For this review, take the finished solid that the model builds, in its own axes (mm). Face numbers are marked on the shaded views. A direction names the side the tool comes from. Give positions to 0.01 mm unless a question says otherwise; leave off trailing zeros. Write each loop counter-clockwise with the first axis right and the second up, starting at its lowest first coordinate (ties: lowest second). Pieces come first, ordered by that corner, then holes.
from build123d import *

# Parameters (mm, degrees)
SKETCH1_W           = 80
SKETCH1_H           = 30
SKETCH1_R           = 5.5
BOSS_EXTRUDE1_DEPTH = 6
SKETCH3_W           = 50
SKETCH3_H           = 30
SKETCH3_R           = 5
BOSS_EXTRUDE2_DEPTH = 6
FILLET1_R           = 2
CHAMFER1_SIZE       = 5


with BuildPart() as part:
    # Sketch1 → Boss-Extrude1 (new body)
    with BuildSketch(Plane.XY):
        Rectangle(SKETCH1_W, SKETCH1_H)
        Circle(SKETCH1_R, mode=Mode.SUBTRACT)
        with Locations((-25, 0)):
            Circle(SKETCH1_R, mode=Mode.SUBTRACT)
    extrude(amount=BOSS_EXTRUDE1_DEPTH)

    # Sketch3 → Boss-Extrude2 (add)
    with BuildSketch(Plane(origin=(40, 0, 0), x_dir=(0, 0, -1), z_dir=(1, 0, 0))):
        with Locations((-25, 0)):
            Rectangle(SKETCH3_W, SKETCH3_H)
        with Locations((-40, 0)):
            Circle(SKETCH3_R, mode=Mode.SUBTRACT)
    extrude(amount=-BOSS_EXTRUDE2_DEPTH)

    # Fillet1
    fillet1_edges = [part.edges().sort_by_distance(p)[0] for p in [
        (34, 0, 6),
        (40, 0, 0),
    ]]
    fillet(fillet1_edges, radius=FILLET1_R)

    # Chamfer1
    chamfer1_edges = [part.edges().sort_by_distance(p)[0] for p in [
        (37, 15, 50),
        (37, -15, 50),
        (-40, -15, 3),
        (-40, 15, 3),
    ]]
    chamfer(chamfer1_edges, length=CHAMFER1_SIZE)


solid = part.part
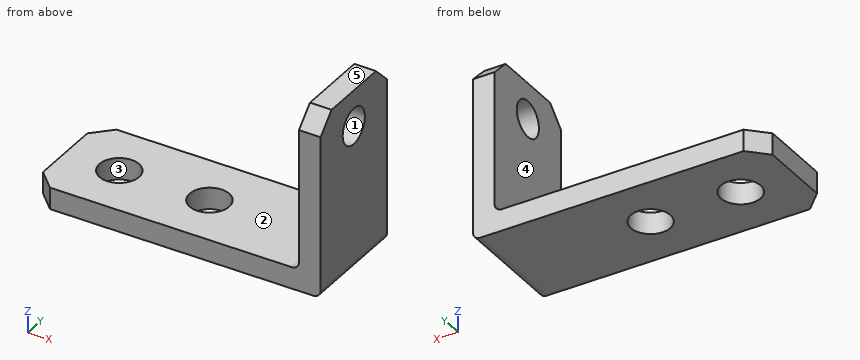
(1) We need section D-D (z = 9). Write out the cut boundary in (x, y), and give its area (3 significant figures).
(2) Tool access review of the marked faces 4 and 5: name each direction out of +Z, -Z, +X, -X, +Y, -Y from which nothing blocks a thin tool from reaching the whole face with its end or side.
(3) Clearance check with flat-ended pins moving along their axes: pin 1 Ø9 at (x, y) = (-9, 5.5) entering from +Z; pin 2 Ø6 at (y, z) = (-11.5, 13) entering from -X; pin 3 Ø4 at (x, y) = (-11, -2.5) entering from -Z; pin 4 Ø9 at (y, z) = (0, 40) entering from -X. State where each tip first meets the part, or that it passes through.
(4) We need section B-B (y = 0). Write out the cut boundary in (x, z).
(5) The part is to be moulded in two halves that separate along Z. For the marked faces 1, 2 and 3, say which applies: +Z half, -Z half, draft (parallel to the pull), parting line (faces both ways), or undercut.
(6) We need section A-A (x = -25). Write out the cut boundary in (y, z), and give its area (3 significant figures).
(7) We need section C-C (z = 40). Write out the cut boundary in (x, y).
(8) For L1, parallel to Y at x = 38.1, z = 40; L2, parallel to Y at x = -25, z = 1.65; L3, parallel to Z at x = -6, y = -2.5, list the stretches that pass through material, from the lowest coordinate up.
The answers:
1. outline: (34, -15) - (40, -15) - (40, 15) - (34, 15) - close
1. area: 180 mm2
2. face 4: +Z, -X, +Y, -Y
2. face 5: +Z, +X, -X, +Y, -Y
3. pin 1: stops at z = 6
3. pin 2: stops at x = 34
3. pin 3: stops at z = 0
3. pin 4: passes through
4. outline: (-40, 0) - (-30.5, 0) - (-30.5, 6) - (-40, 6) - close; (-19.5, 0) - (-5.5, 0) - (-5.5, 6) - (-19.5, 6) - close; (5.5, 0) - (38, 0) arc R2 ccw to (40, 2) - (40, 35) - (34, 35) - (34, 8) arc R2 cw to (32, 6) - (5.5, 6) - close; (34, 45) - (40, 45) - (40, 50) - (34, 50) - close
5. face 1: undercut
5. face 2: +Z half
5. face 3: draft
6. outline: (-15, 0) - (-5.5, 0) - (-5.5, 6) - (-15, 6) - close; (5.5, 0) - (15, 0) - (15, 6) - (5.5, 6) - close
6. area: 114 mm2
7. outline: (34, -15) - (40, -15) - (40, -5) - (34, -5) - close; (34, 5) - (40, 5) - (40, 15) - (34, 15) - close
8. L1: y = -15 to -5, 5 to 15
8. L2: y = -15 to -5.5, 5.5 to 15
8. L3: z = 0 to 6
